Read the model definition and answer for the solid it produces. Units are mm, in the model's axes. Face numbers are marked on the shaded views. A direction names the side the tool comes from. Coordinates: 2 decimals unless noted, no trailing zeros. Write each loop counter-clockwise with the first axis right and the second up, starting at its lowest first coordinate (ties: lowest second). Pieces come first, ordered by that corner, then holes. Notation, with made-up numbers: (66.5, 29.25) -> (122.5, 29.25) arc R24 ccw to (122.5, 42.25) -> close; hole circle Ø7 at (6.5, 1.5). An arc over 180 degrees is marked (long way). Answer in a Markdown table with one row per item. Add a question column.
Item 1: For a pull along Y with two mould halves and no side action, classify the marked faces 1, 2 and 3 as +Y half, -Y half, draft (parallel to the pull), parting line (faces both ways), or undercut.
Item 2: Given pin 1 Ø1 at (x, z) = (-2.5, -3) entering from -Y; pin 2 Ø5 at (x, z) = (3, -13) entering from -Y; pin 3 Ø1 at (x, y) = (2.5, 1.5) entering from -Z, each flat-ended and moving along its own axis, determine where each tip first touches the part or whether it passes through.
Item 3: Straight lines are drawn through the part: line 1 (X direction, y = -2, z = 4.25); line 2 (Z direction, x = -1.75, y = 3.75); line 3 (Z direction, x = 1.5, y = 1.75). For each, find the intervals that lie inside material, in ascending order. Write a range as from..to.
Item 4: Section A-A on z = -14.75 is taken. Write down the section's boundary in (x, y), then the cut area to 3 significant figures.
Item 5: Which of the six approach directions +Z, -Z, +X, -X, +Y, -Y give full straight-line access (tool end or side, diameter ignored) to the marked faces 4 and 5?
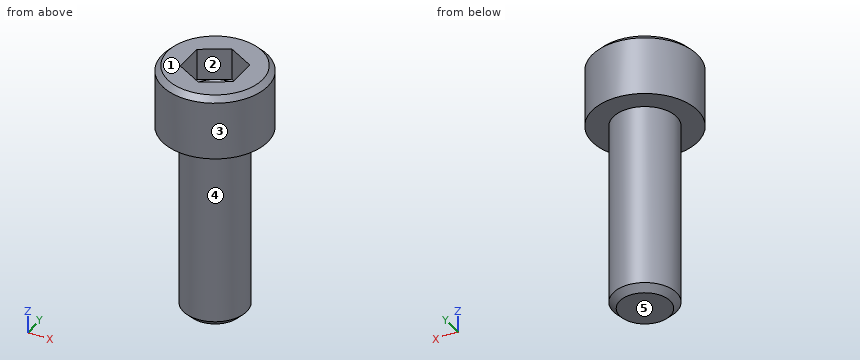
```python
from build123d import *

# Parameters (mm, degrees)
SKETCH_1_W          = 5
SKETCH_1_H          = 6
SKETCH_2_R          = 3
EXTRUDE_1_DEPTH     = 18
CUT_EXTRUDE_1_DEPTH = 3
CHAMFER_1_SIZE      = 0.5
CHAMFER_2_SIZE      = 0.6135


with BuildPart() as part:
    # 草图1 → 旋转1 (revolve)
    with BuildSketch(Plane(origin=(0, 0, 0), x_dir=(1, 0, 0), z_dir=(0, 1, 0))):
        with Locations((2.5, -3)):
            Rectangle(SKETCH_1_W, SKETCH_1_H)
    revolve(axis=Axis((0, 0, 0), (0, 0, 1)))

    # 草图2 → 凸台-拉伸1 (add)
    with BuildSketch(Plane(origin=(0, 0, 0), x_dir=(-1, 0, 0), z_dir=(0, 0, -1))):
        Circle(SKETCH_2_R)
    extrude(amount=EXTRUDE_1_DEPTH)

    # 草图3 → 切除-拉伸1 (cut)
    with BuildSketch(Plane.XY.offset(6)):
        Polygon((2.5, 1.443375673), (0, 2.886751346), (-2.5, 1.443375673), (-2.5, -1.443375673), (0, -2.886751346), (2.5, -1.443375673), align=None)
    extrude(amount=-CUT_EXTRUDE_1_DEPTH, mode=Mode.SUBTRACT)

    # 草图4 → 切除-旋转1 (revolve, cut)
    with BuildSketch(Plane.XZ):
        Polygon((2.5, 3), (0, 3), (0, 1.556624327), align=None)
    revolve(axis=Axis((0, 0, 3), (0, 0, -1)), mode=Mode.SUBTRACT)

    # 倒角1
    chamfer_1_edges = [part.edges().sort_by_distance(p)[0] for p in [
        (-5, 0, 6),
    ]]
    chamfer(chamfer_1_edges, length=CHAMFER_1_SIZE)

    # 倒角2
    chamfer_2_edges = [part.edges().sort_by_distance(p)[0] for p in [
        (3, 0, -18),
    ]]
    chamfer(chamfer_2_edges, length=CHAMFER_2_SIZE)


solid = part.part
```
Results below:
| question | item | result |
|---|---|---|
| 1 | face 1 | draft |
| 1 | face 2 | undercut |
| 1 | face 3 | parting line |
| 2 | pin 1 | stops at y = -2.24 |
| 2 | pin 2 | stops at y = -2.96 |
| 2 | pin 3 | stops at z = -17.97 |
| 3 | line 1 | x = -4.58..-1.54, 1.54..4.58 |
| 3 | line 2 | z = 0..6 |
| 3 | line 3 | z = -18..2.89 |
| 4 | outline | circle Ø6 at (0, 0) |
| 4 | area | 28.3 mm2 |
| 5 | face 4 | -Z |
| 5 | face 5 | -Z, +X, -X, +Y, -Y |
